CAD build for the part. Positions are in the model's coordinates, mm. A direction names the side the tool comes from. Coordinates: 2 decimals unless noted, no trailing zeros. Order: outer loops, then holes, each group sorted by start corner. A loop starts at its lowest first (then second) coordinate and runs counter-clockwise, first axis right, second up. Notation, with made-up numbers: M 20.5,26.5 L 59.5,26.5 A18 cw 59.5,56.5 Z; hole C 73,72 d8. An arc over 180 degrees is marked long. One line per item, written item: value.
from build123d import *

# Parameters (mm, degrees)
SKETCH2_OUTSIDE_W  = 31.222
SKETCH2_OUTSIDE_H  = 31.222
CUT_EXTRUDE2_DEPTH = 10
SCALE_1_SCALE      = 1.875


with BuildPart() as part:
    # Sketch1 → Revolve1 (revolve)
    with BuildSketch(Plane.XY, mode=Mode.PRIVATE) as revolve1_sk:
        Polygon((0, 0), (9, 0), (9, 9), (5, 9), (5, 49), (4, 50), (0, 50), align=None)
    revolve(revolve1_sk.sketch.rotate(Axis((0, 50, 0), (0, -1, 0)), 90), axis=Axis((0, 50, 0), (0, -1, 0)))

    # Sketch2 outside → Cut-Extrude2 (cut)
    with BuildSketch(Plane.XZ):
        Rectangle(SKETCH2_OUTSIDE_W, SKETCH2_OUTSIDE_H)
        Polygon((9, 0), (4.5, 7.794228634), (-4.5, 7.794228634), (-9, 0), (-4.5, -7.794228634), (4.5, -7.794228634), align=None, mode=Mode.SUBTRACT)
    extrude(amount=-CUT_EXTRUDE2_DEPTH, mode=Mode.SUBTRACT)

    # Sketch5 → Cut-Revolve2 (revolve, cut)
    with BuildSketch(Plane.XY, mode=Mode.PRIVATE) as cut_revolve2_sk:
        with BuildLine():
            Line((-9, 0), (-9, 1))
            ThreePointArc((-9, 1), (-8.071297978, 0.357404043), (-7, 0))
            Line((-7, 0), (-9, 0))
        make_face()
    revolve(cut_revolve2_sk.sketch.rotate(Axis((0, 0, 0), (0, 1, 0)), 270), axis=Axis((0, 0, 0), (0, 1, 0)), mode=Mode.SUBTRACT)


with BuildPart() as part_1:
    # Scale 1: scaled about (-2.65e-07, 20.203740947, 0)
    add(part.part.scale(SCALE_1_SCALE).moved(Location((2.32e-07, -17.678273329, 0))))


solid = part_1.part
Q1. Which spindle directions (+Z, -Z, +X, -X, +Y, -Y) get a long thin tool onto all of the face, cutting with end or side? Do faces 4 (the face through (-12.72, -9.14, -7.2)), 5 (the face through (-9.295, 37.222, -1.22)). Say none if no direction does.
Recorded:
face 4: -Z, -X, +Y, -Y
face 5: +Y
Q2. Drill centre lines: line 1 along Y through (x, z) = (-0.5, 12); line 2 along Z through (x, y) = (-0.5, 35.5); line 3 along X through (y, z) = (-6, -13). Where is each one in solid material? Low to high.
Recorded:
line 1: y = -17.68 to -0.8
line 2: z = -9.36 to 9.36
line 3: x = -9.37 to 9.37
Q3. Slice it at A-A (y = 59). List the corners of the cut face in (x, z) (3 decimals), plus the area to 3 significant figures.
Recorded:
outline: C 0,0 d18.75
area: 276 mm^2
Q4. Mould opens along X. For faces 1 (the face through (0, -17.678, 0)), 2 (the face through (12.72, -9.14, 7.2)), 3 (the face through (-12.597, -9.139, 7.409)) say: released by +X, released by -X, zero draft, split by the parting line, or undercut.
Recorded:
face 1: zero draft
face 2: released by +X
face 3: released by -X
Q5. Pin check, flat tips, straight feed: pin 1 Ø12 at (x, y) = (-1, 55.5) entering from -Z (3 decimals); pin 2 Ø4 at (y, z) = (4.5, 3.5) entering from +X; pin 3 Ø3 at (x, z) = (-9.5, 5) entering from +Y; pin 4 Ø12 at (x, z) = (-10.5, -7) entering from +Y. Stop position of each tip, or through.
Recorded:
pin 1: stops at z = -9.375
pin 2: stops at x = 9.25
pin 3: stops at y = 74.34
pin 4: stops at y = 76.07
